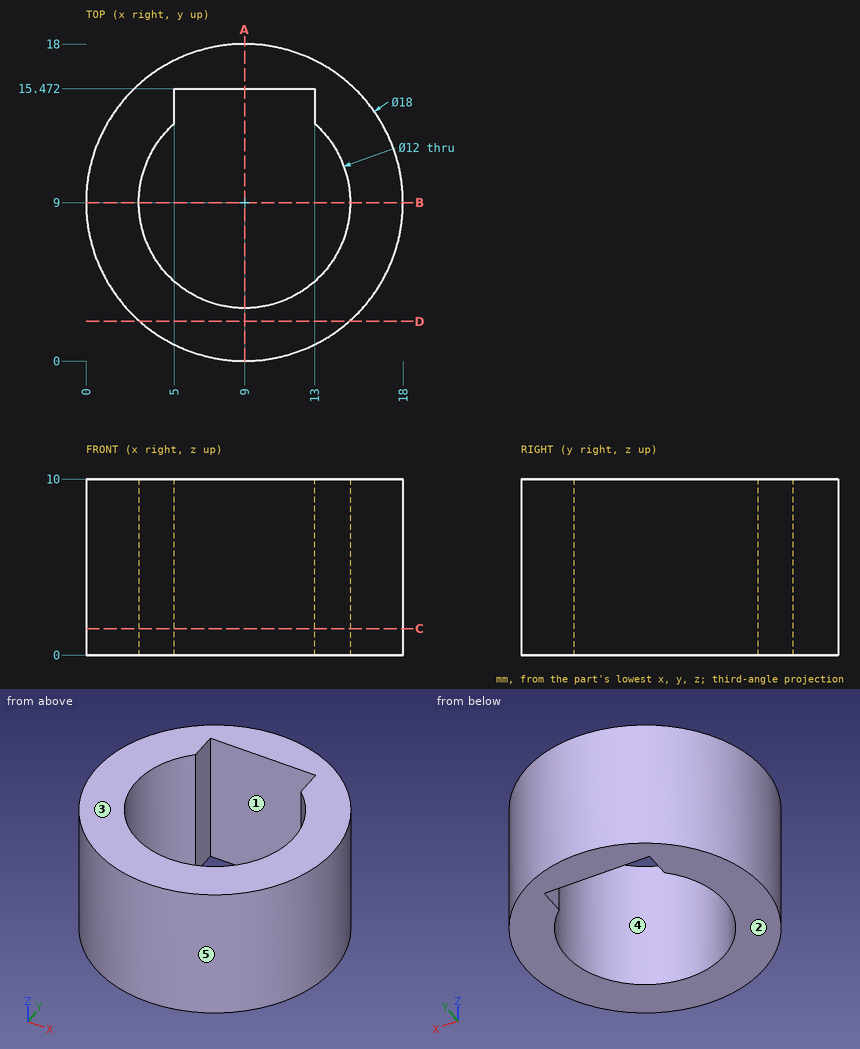
Drawing for the job (mm, zero at the part's lowest x, y, z). A direction names the side the tool comes from. Coordinates: 2 decimals unless noted, no trailing zeros. Write each loop counter-clockwise with the first axis right and the second up, starting at its lowest first coordinate (ties: lowest second). Pieces come first, ordered by that corner, then holes. Notation, with made-up numbers: (46.5, 66.25) -> (95.5, 66.25) arc R29 cw to (95.5, 86.25) -> close; hole circle Ø6 at (-21.5, 9.5). An arc over 180 degrees is marked (long way). One line per item, written item: value. Start each with the question number.
1) Flat gauge pins, fed straight in: pin 1 Ø2.5 at (x, z) = (11, 3) entering from -Y; pin 2 Ø0.6 at (y, z) = (15, 4.5) entering from +X (1 decimal); pin 3 Ø1.6 at (y, z) = (14, 5.5) entering from -X. Where does each tip first touch, or does it go through?
2) Slice it at D-D on y = 2.25. Write the cut outline in (x, z), then the cut area to 3 significant figures.
3) Pull direction X, two halves, no side cores. Call the marked faces 3, 4 and 5: +X half, -X half, draft (parallel to the pull), parting line (faces both ways), or undercut.
4) Probe probe 1 along Y at (x, z) = (9, 3); probe 2 along X at (y, z) = (8.75, 4.5) (1 decimal); probe 3 along Y at (x, z) = (8, 3). List the from-to ranges inside material, lowest first.
5) Which spindle directions (+Z, -Z, +X, -X, +Y, -Y) get a long thin tool onto all of the face, cutting with end or side? Do the marked faces 1 and 2. Say none if no direction does.
6) Slice it at A-A on x = 9. Write the cut outline in (y, z), then the cut area to 3 significant figures.
7) Slice it at B-B on y = 9. Write the cut outline in (x, z).
8) Slice it at C-C on z = 1.5. Write the cut outline in (x, y), then the cut area to 3 significant figures.
Answers follow:
1. pin 1: y = 0.03
1. pin 2: x = 16
1. pin 3: x = 1.04
2. outline: (3.05, 0) -> (14.95, 0) -> (14.95, 10) -> (3.05, 10) -> close
2. area: 119 mm2
3. face 3: draft
3. face 4: undercut
3. face 5: parting line
4. probe 1: 0 to 3, 15.47 to 18
4. probe 2: 0 to 3, 15 to 18
4. probe 3: 0.06 to 3.08, 15.47 to 17.94
5. face 1: +Z, -Z
5. face 2: -Z, +X, -X, +Y, -Y
6. outline: (0, 0) -> (3, 0) -> (3, 10) -> (0, 10) -> close; (15.47, 0) -> (18, 0) -> (18, 10) -> (15.47, 10) -> close
6. area: 55.3 mm2
7. outline: (0, 0) -> (3, 0) -> (3, 10) -> (0, 10) -> close; (15, 0) -> (18, 0) -> (18, 10) -> (15, 10) -> close
8. outline: circle Ø18 at (9, 9); hole (5, 13.47) arc R6 ccw (long way) to (13, 13.47) -> (13, 15.47) -> (5, 15.47) -> close
8. area: 134 mm2
